from build123d import *

# Parameters (mm, degrees)
BASE_EXTRUDE_DEPTH      = 0.5
BASE_EXTRUDE_DEPTH_BACK = 0.5
SKETCH1_R               = 0.85


with BuildPart() as part:
    # Sketch1 → Base-Extrude (new, two sides: drawn at the far end of the back side and taken through both)
    with BuildSketch(Plane.XY.offset(-BASE_EXTRUDE_DEPTH_BACK)):
        with BuildLine():
            Line((-1, -7.861655032), (-1, -11.584658105))
            ThreePointArc((-1, -11.584658105), (-2.996355114, -11.21599342), (-4.89157372, -10.488330159))
            ThreePointArc((-4.89157372, -10.488330159), (-4.963053699, -10.428973531), (-5, -10.343723502))
            Line((-5, -10.343723502), (-5.51947234, -7.397649464))
            ThreePointArc((-5.51947234, -7.397649464), (-5.581565084, -7.229851618), (-5.698757664, -7.094657221))
            ThreePointArc((-5.698757664, -7.094657221), (0, 9.1), (5.698757664, -7.094657221))
            ThreePointArc((5.698757664, -7.094657221), (5.581565084, -7.229851618), (5.51947234, -7.397649464))
            Line((5.51947234, -7.397649464), (5, -10.343723502))
            ThreePointArc((5, -10.343723502), (4.963053699, -10.428973531), (4.89157372, -10.488330159))
            ThreePointArc((4.89157372, -10.488330159), (2.996355114, -11.21599342), (1, -11.584658105))
            Line((1, -11.584658105), (1, -7.861655032))
            ThreePointArc((1, -7.861655032), (0, 6.77), (-1, -7.861655032))
        make_face()
        with Locations((-3, -9.277125962)):
            Circle(SKETCH1_R, mode=Mode.SUBTRACT)
        with Locations(Location((3, -9.277125962, 0), (0, 0, 180))):
            Circle(SKETCH1_R, mode=Mode.SUBTRACT)
    extrude(amount=BASE_EXTRUDE_DEPTH + BASE_EXTRUDE_DEPTH_BACK)


solid = part.part
The model under review builds one solid part; all positions refer to its coordinate system, in mm. A direction names the side the tool comes from. Round coordinates to 2 decimals unless told otherwise and drop trailing zeros. Order: outer loops, then holes, each group sorted by start corner. A loop starts at its lowest first (then second) coordinate and runs counter-clockwise, first axis right, second up. Notation, with made-up numbers: (32.5, 15) -> (88.5, 15) arc R14 ccw to (88.5, 35) -> close; hole circle Ø5 at (88, 10.25). An arc over 180 degrees is marked (long way). Write item = value, one per line. Start each with the question number.
Item 1: For line 1 along X through (y, z) = (-9, 0.25); line 2 along Y through (x, z) = (-2.25, 0.25); line 3 along X through (y, z) = (-8.75, 0.4), list the stretches that pass through material, from the lowest coordinate up.
Item 2: Clearance check with a flat-ended pin moving along its axis: pin 1 Ø1 at (x, y) = (-2, -5) entering from +Z. State where the tip first meets the part, or that it passes through.
Item 3: Mouldability with a two-part tool opening along X and no side actions: class faces 3 (the face through (1, -10, 0)), 4 (the face through (-0.314, 9.095, -0.007)), 5 (the face through (3.02, -11.21, -0.01)) as released by +X, released by -X, zero draft, split by the parting line, or undercut.
Item 4: Consider section D-D on x = 0. Write out the cut boundary in (y, z), plus the area to 3 significant figures.
Item 5: Consider section C-C on z = -0.1. Write out the cut boundary in (x, y).
Item 6: Consider section A-A on y = -0.58. Write out the cut boundary in (x, z), plus the area to 3 significant figures.
Item 7: Consider section B-B on x = -3. Write out the cut boundary in (y, z), plus the area to 3 significant figures.
Item 8: For faces 1 (the face through (-1, -10, 0)), 2 (the face through (-2.969, -11.224, -0.007)), list the 3-axis set-ups (+Z, -Z, +X, -X, +Y, -Y) from which the entire face can be reached by the end or side of a thin tool; tool diameter is ignored.
Conclusion:
q1.line_1 = -5.24 to -3.8, -2.2 to -1, 1 to 2.2, 3.8 to 5.24
q1.line_2 = -11.4 to -9.68, -8.88 to -7.58, 6.42 to 8.82
q1.line_3 = -5.28 to -3.67, -2.33 to -1, 1 to 2.33, 3.67 to 5.28
q2.pin_1 = through
q3.face_3 = undercut
q3.face_4 = split by the parting line
q3.face_5 = released by +X
q4.outline = (6.77, -0.5) -> (9.1, -0.5) -> (9.1, 0.5) -> (6.77, 0.5) -> close
q4.area = 2.33 mm2
q5.outline = (-5.7, -7.09) arc R0.5 cw to (-5.52, -7.4) -> (-5, -10.34) arc R0.2 ccw to (-4.89, -10.49) arc R11.05 ccw to (-1, -11.58) -> (-1, -7.86) arc R7.35 cw (long way) to (1, -7.86) -> (1, -11.58) arc R11.05 ccw to (4.89, -10.49) arc R0.2 ccw to (5, -10.34) -> (5.52, -7.4) arc R0.5 cw to (5.7, -7.09) arc R9.1 ccw (long way) to start; hole circle Ø1.7 at (-3, -9.28); hole circle Ø1.7 at (3, -9.28)
q6.outline = (-9.08, -0.5) -> (-7.35, -0.5) -> (-7.35, 0.5) -> (-9.08, 0.5) -> close; (7.35, -0.5) -> (9.08, -0.5) -> (9.08, 0.5) -> (7.35, 0.5) -> close
q6.area = 3.46 mm2
q7.outline = (-11.21, -0.5) -> (-10.13, -0.5) -> (-10.13, 0.5) -> (-11.21, 0.5) -> close; (-8.43, -0.5) -> (-7.29, -0.5) -> (-7.29, 0.5) -> (-8.43, 0.5) -> close; (6.13, -0.5) -> (8.59, -0.5) -> (8.59, 0.5) -> (6.13, 0.5) -> close
q7.area = 4.69 mm2
q8.face_1 = +Z, -Z, -Y
q8.face_2 = +Z, -Z, -X, -Y
